Could you check a few things on this drawing? It's one solid part, dimensions in mm from its lowest x, y, z. A direction names the side the tool comes from. Give positions to 0.01 mm unless a question says otherwise; leave off trailing zeros. Order: outer loops, then holes, each group sorted by start corner. A loop starts at its lowest first (then second) coordinate and runs counter-clockwise, first axis right, second up. Notation, with made-up numbers: (68.5, 27.25) -> (84.5, 27.25) arc R21 ccw to (84.5, 45.25) -> close; hole circle Ø10 at (72.25, 5). An arc over 180 degrees is marked (long way). Answer as CSV lines item,"result".
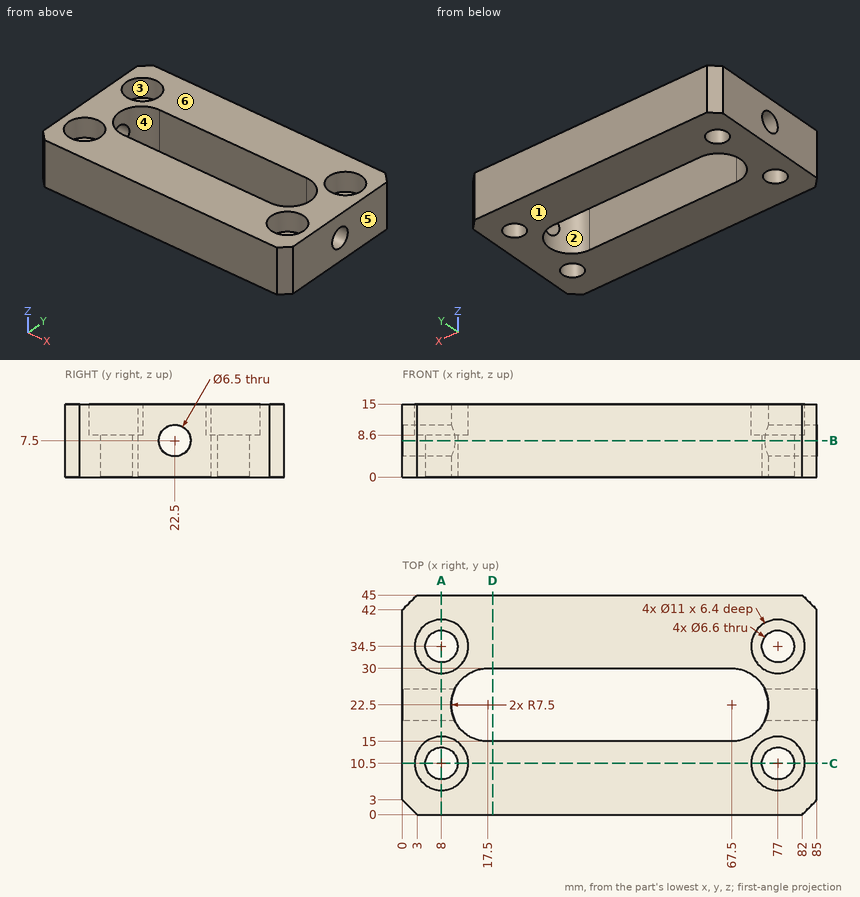
Item 1: For pin 1 (9 mm diameter, centred on x = 77, y = 34.5, fed in from +Z); pin 2 (4 mm diameter, centred on x = 13.5, y = 23.5, fed in from +Z), each with a flat end and sliding along its axis, tell me the tip position at first contact or that it passes through.
Numbers:
pin 1,"stops at z = 8.6"
pin 2,"passes through"
Item 2: For the marked faces 1, 2 and 3, which set-ups out of +Z, -Z, +X, -X, +Y, -Y let a thin tool reach every point of the face, with its end or its side?
Numbers:
face 1,"-Z, +X, -X, +Y, -Y"
face 2,"+Z, -Z"
face 3,"+Z"
Item 3: Imagine slicing it at B-B, the plane z = 7.5. Please give me the cut outline in (x, y), then the cut area to 3 significant figures.
Numbers:
outline,"(0, 3) -> (3, 0) -> (82, 0) -> (85, 3) -> (85, 19.25) -> (74.26, 19.25) arc R7.5 cw to (67.5, 15) -> (17.5, 15) arc R7.5 cw to (10.74, 19.25) -> (0, 19.25) -> close; (0, 25.75) -> (10.74, 25.75) arc R7.5 cw to (17.5, 30) -> (67.5, 30) arc R7.5 cw to (74.26, 25.75) -> (85, 25.75) -> (85, 42) -> (82, 45) -> (3, 45) -> (0, 42) -> close; hole circle Ø6.6 at (8, 10.5); hole circle Ø6.6 at (8, 34.5); hole circle Ø6.6 at (77, 10.5); hole circle Ø6.6 at (77, 34.5)"
area,"2,610 mm²"
Item 4: Please list where these lines run through material, in increasing order: line 1 along Y through (x, z) = (77, 2.25); line 2 along Y through (x, z) = (77, 11); line 3 along Y through (x, z) = (25.5, 11).
Numbers:
line 1,"y = 0 to 7.2, 13.8 to 31.2, 37.8 to 45"
line 2,"y = 0 to 5, 16 to 29, 40 to 45"
line 3,"y = 0 to 15, 30 to 45"
Item 5: Imagine slicing it at C-C, the plane y = 10.5. Please give me the cut outline in (x, z), then the cut area to 3 significant figures.
Numbers:
outline,"(0, 0) -> (4.7, 0) -> (4.7, 8.6) -> (2.5, 8.6) -> (2.5, 15) -> (0, 15) -> close; (11.3, 0) -> (73.7, 0) -> (73.7, 8.6) -> (71.5, 8.6) -> (71.5, 15) -> (13.5, 15) -> (13.5, 8.6) -> (11.3, 8.6) -> close; (80.3, 0) -> (85, 0) -> (85, 15) -> (82.5, 15) -> (82.5, 8.6) -> (80.3, 8.6) -> close"
area,"1,020 mm²"
Item 6: Imagine slicing it at A-A, the plane x = 8. Please give me the cut outline in (y, z), then the cut area to 3 significant figures.
Numbers:
outline,"(0, 0) -> (7.2, 0) -> (7.2, 8.6) -> (5, 8.6) -> (5, 15) -> (0, 15) -> close; (13.8, 0) -> (31.2, 0) -> (31.2, 8.6) -> (29, 8.6) -> (29, 15) -> (16, 15) -> (16, 8.6) -> (13.8, 8.6) -> close; (37.8, 0) -> (45, 0) -> (45, 15) -> (40, 15) -> (40, 8.6) -> (37.8, 8.6) -> close; hole circle Ø6.5 at (22.5, 7.5)"
area,"387 mm²"
Item 7: Imagine slicing it at D-D, the plane x = 18.5. Please give me the cut outline in (y, z), then the cut area to 3 significant figures.
Numbers:
outline,"(0, 0) -> (15, 0) -> (15, 15) -> (0, 15) -> close; (30, 0) -> (45, 0) -> (45, 15) -> (30, 15) -> close"
area,"450 mm²"
Item 8: We'd pull the mould along X, two halves only. Please class the marked faces 4, 5 and 6: released by +X, released by -X, zero draft, split by the parting line, or undercut.
Numbers:
face 4,"undercut"
face 5,"released by +X"
face 6,"zero draft"
